Geometry check sheet. Reference: the model listing, model coordinates, mm. A direction names the side the tool comes from. Round coordinates to 2 decimals unless told otherwise and drop trailing zeros. Loops run counter-clockwise (first coordinate to the right, second up) from the corner with the lowest first, then second, coordinate; pieces in that order, holes last. Notation, with made-up numbers: M 27.25,-4.75 L 40.25,-4.75 A17 cw 40.25,28.25 Z; hole C 1.5,-36 d10. An arc over 180 degrees is marked long. Use one line per item in the form item = value. Start each with the question number.
1. Cross-section at B-B (x = 10.5). State how many separate pieces and enclosed holes the cut face has, then the cut area to 3 significant figures.
2. Set-up check for faces 1 (the cylindrical face through (10.563, -12.797, 35.846)), 2 (the cylindrical face through (8, 5, 46)): record each of +Z, -Z, +X, -X, +Y, -Y from which the full face is reachable in a straight line by a thin tool's end or side.
3. Material ranges on line 1 (Z direction, x = 8.5, y = 27.55); line 2 (Z direction, x = 6, y = 4.95); line 3 (Y direction, x = 8, z = 3), recorded low to high.
4. Go/stop test with flat-tipped pins: pin 1 (2.5 mm diameter, centred on y = -107.55, z = -94, fed in from +X); pin 2 (7.5 mm diameter, centred on x = 5, z = 51.5, fed in from -Y); pin 3 (7.5 mm diameter, centred on y = -18, z = 42.5, fed in from +X). Record where each tip stops, or that it passes through.
5. Draft check along Z on faces 3 (the flat face through (7, 0, 104)), 4 (the flat face through (7, -35.05, 24)), 5 (the cylindrical face through (10.94, -105.07, -79.33)). Enter one of: pulls with the +Z half, pulls with the -Z half, needs draft (parallel to the pull), parting line crosses it, or undercut.
6. Cross-section at C-C (y = -69.5). Record the boundary of the cut face in (x, z), then the cut area to 3 significant figures.
7. Cross-section at A-A (z = -67). Record the boundary of the cut face in (x, y), then the cut area to 3 significant figures.
```python
from build123d import *

# Parameters (mm, degrees)
SKETCH1_W                                            = 208
SKETCH1_H                                            = 70.1
BOSS_EXTRUDE1_DEPTH                                  = 15
CBORE_FOR_M8_HEXAGON_SOCKET_HEAD_CAP_SCR_D           = 9
CBORE_FOR_M8_HEXAGON_SOCKET_HEAD_CAP_SCR_CBORE_D     = 15
CBORE_FOR_M8_HEXAGON_SOCKET_HEAD_CAP_SCR_CBORE_DEPTH = 9
F_6_0MM_BLIND_HOLE_1_AT_2_COUNT                      = 2
F_6_0MM_BLIND_HOLE_1_AT_2_PITCH                      = 40
SKETCH6_W                                            = 15
SKETCH6_H                                            = 44
BOSS_EXTRUDE2_DEPTH                                  = 82
M5_TAPPED_HOLE1_D                                    = 4.2
M5_TAPPED_HOLE1_DEPTH                                = 12.4
M5_TAPPED_HOLE1_TIP                                  = 1.2618073
F_5_0MM_BLIND_HOLE_1_D                               = 5
F_5_0MM_BLIND_HOLE_1_DEPTH                           = 8
F_5_0MM_BLIND_HOLE_1_TIP                             = 1.502151548
M6_TAPPED_HOLE1_D                                    = 5
M6_TAPPED_HOLE1_DEPTH                                = 15
M6_TAPPED_HOLE1_TIP                                  = 1.502151548
F_5_0MM_BLIND_HOLE_2_D                               = 5
F_5_0MM_BLIND_HOLE_2_DEPTH                           = 8
F_5_0MM_BLIND_HOLE_2_TIP                             = 1.502151548
M5_TAPPED_HOLE2_D                                    = 4.2
M5_TAPPED_HOLE2_DEPTH                                = 12.4
M5_TAPPED_HOLE2_TIP                                  = 1.2618073
M8_CLEARANCE_HOLE1_D                                 = 9
F_6_0MM_BLIND_HOLE_2_D                               = 6
FILLET1_R                                            = 5
CHAMFER1_SIZE                                        = 3


with BuildPart() as part:
    # Sketch1 → Boss-Extrude1 (new body)
    with BuildSketch(Plane(origin=(0, 0, 0), x_dir=(0, 0, -1), z_dir=(1, 0, 0))):
        Rectangle(SKETCH1_W, SKETCH1_H)
    extrude(amount=BOSS_EXTRUDE1_DEPTH)

    # CBORE for M8 Hexagon socket head cap screws1 (through all)
    with Locations(Plane(origin=(15, 0, 0), x_dir=(0, 0, -1), z_dir=(1, 0, 0))):
        with Locations((-43, -15.05), (-3, -15.05)):
            CounterBoreHole(CBORE_FOR_M8_HEXAGON_SOCKET_HEAD_CAP_SCR_D / 2, CBORE_FOR_M8_HEXAGON_SOCKET_HEAD_CAP_SCR_CBORE_D / 2, CBORE_FOR_M8_HEXAGON_SOCKET_HEAD_CAP_SCR_CBORE_DEPTH)

    # Sketch5 → Ø6.0mm blind hole 1 (revolve, cut)
    with BuildSketch(Plane(origin=(15, 4.95, 43), x_dir=(0, 0, -1), z_dir=(0, 1, 0))):
        Polygon((0, 0), (0, 15), (3.25, 15), (3, 14.75), (3, 0.25), (3.25, 0), align=None)
    f_6_0mm_blind_hole_1 = revolve(axis=Axis((21.35, 4.95, 43), (-1, 0, 0)), mode=Mode.SUBTRACT)

    # Ø6.0mm blind hole 1 at 2: Ø6.0mm blind hole 1 ×2
    with Locations(*[(0, 0, -i * F_6_0MM_BLIND_HOLE_1_AT_2_PITCH) for i in range(1, F_6_0MM_BLIND_HOLE_1_AT_2_COUNT)]):
        add(f_6_0mm_blind_hole_1, mode=Mode.SUBTRACT)

    # Sketch6 → Boss-Extrude2 (add)
    with BuildSketch(Plane.XZ.offset(35.05)):
        with Locations((7.5, -82)):
            Rectangle(SKETCH6_W, SKETCH6_H)
    extrude(amount=BOSS_EXTRUDE2_DEPTH)

    # M5 Tapped Hole1
    with Locations(Plane(origin=(15, 0, 0), x_dir=(0, 0, -1), z_dir=(1, 0, 0))):
        with Locations((94, -107.55), (94, -52.55)):
            Hole(M5_TAPPED_HOLE1_D / 2, depth=M5_TAPPED_HOLE1_DEPTH)
            with Locations((0, 0, -(M5_TAPPED_HOLE1_DEPTH + M5_TAPPED_HOLE1_TIP / 2))):  # 118° drill point
                Cone(0, M5_TAPPED_HOLE1_D / 2, M5_TAPPED_HOLE1_TIP, mode=Mode.SUBTRACT)

    # Ø5.0mm blind hole 1
    with Locations(Plane(origin=(15, 0, 0), x_dir=(0, 0, -1), z_dir=(1, 0, 0))):
        with Locations((79, -52.55), (79, -107.55)):
            Hole(F_5_0MM_BLIND_HOLE_1_D / 2, depth=F_5_0MM_BLIND_HOLE_1_DEPTH)
            with Locations((0, 0, -(F_5_0MM_BLIND_HOLE_1_DEPTH + F_5_0MM_BLIND_HOLE_1_TIP / 2))):  # 118° drill point
                Cone(0, F_5_0MM_BLIND_HOLE_1_D / 2, F_5_0MM_BLIND_HOLE_1_TIP, mode=Mode.SUBTRACT)

    # M6 Tapped Hole1
    with Locations(Plane(origin=(15, 0, 0), x_dir=(0, 0, -1), z_dir=(1, 0, 0))):
        with Locations((-76.5, 27.55), (-36.5, 27.55)):
            Hole(M6_TAPPED_HOLE1_D / 2, depth=M6_TAPPED_HOLE1_DEPTH)
            with Locations((0, 0, -(M6_TAPPED_HOLE1_DEPTH + M6_TAPPED_HOLE1_TIP / 2))):  # 118° drill point
                Cone(0, M6_TAPPED_HOLE1_D / 2, M6_TAPPED_HOLE1_TIP, mode=Mode.SUBTRACT)

    # Ø5.0mm blind hole 2
    with Locations(Plane(origin=(15, 0, 0), x_dir=(0, 0, -1), z_dir=(1, 0, 0))):
        with Locations((-96.5, 27.55), (-16.5, 27.55)):
            Hole(F_5_0MM_BLIND_HOLE_2_D / 2, depth=F_5_0MM_BLIND_HOLE_2_DEPTH)
            with Locations((0, 0, -(F_5_0MM_BLIND_HOLE_2_DEPTH + F_5_0MM_BLIND_HOLE_2_TIP / 2))):  # 118° drill point
                Cone(0, F_5_0MM_BLIND_HOLE_2_D / 2, F_5_0MM_BLIND_HOLE_2_TIP, mode=Mode.SUBTRACT)

    # M5 Tapped Hole2
    with Locations(Plane(origin=(15, 0, 0), x_dir=(0, 0, -1), z_dir=(1, 0, 0))):
        with Locations((-96.5, 2.05), (-16.5, 2.05)):
            Hole(M5_TAPPED_HOLE2_D / 2, depth=M5_TAPPED_HOLE2_DEPTH)
            with Locations((0, 0, -(M5_TAPPED_HOLE2_DEPTH + M5_TAPPED_HOLE2_TIP / 2))):  # 118° drill point
                Cone(0, M5_TAPPED_HOLE2_D / 2, M5_TAPPED_HOLE2_TIP, mode=Mode.SUBTRACT)

    # M8 Clearance Hole1 (through all)
    with Locations(Plane(origin=(15, 0, 0), x_dir=(0, 0, -1), z_dir=(1, 0, 0))):
        with Locations((67, -30.05), (97, -30.05), (67, 19.95), (97, 19.95)):
            Hole(M8_CLEARANCE_HOLE1_D / 2)

    # Ø6.0mm blind hole 2 (through all)
    with Locations(Plane(origin=(15, 0, 0), x_dir=(0, 0, -1), z_dir=(1, 0, 0))):
        with Locations((82, -30.05), (82, 19.95)):
            Hole(F_6_0MM_BLIND_HOLE_2_D / 2)

    # Fillet1
    fillet1_edges = [part.edges().sort_by_distance(p)[0] for p in [
        (7.5, -35.05, -60),
    ]]
    fillet(fillet1_edges, radius=FILLET1_R)

    # Chamfer1
    chamfer1_edges = [part.edges().sort_by_distance(p)[0] for p in [
        (7.5, -117.05, -104),
        (7.5, -117.05, -60),
        (7.5, -35.05, 104),
        (7.5, 35.05, 104),
        (7.5, 35.05, -104),
    ]]
    chamfer(chamfer1_edges, length=CHAMFER1_SIZE)


solid = part.part
```
Reported:
q1.separate_pieces = 1
q1.enclosed_holes = 20
q1.area = 17,300 mm²
q2.face_1 = +X
q2.face_2 = +X, -X
q3.line_1 = -104 to 14, 19 to 34, 39 to 74, 79 to 94, 99 to 104
q3.line_2 = -104 to 0, 6 to 40, 46 to 104
q3.line_3 = -35.05 to -22.55, -7.55 to 1.95, 7.95 to 35.05
q4.pin_1 = 2.09
q4.pin_2 = -35.05
q4.pin_3 = 6
q5.face_3 = pulls with the +Z half
q5.face_4 = needs draft
q5.face_5 = undercut
q6.outline = M 0,-104 L 15,-104 L 15,-60 L 0,-60 Z
q6.area = 660 mm²
q7.outline = M 0,-117.05 L 15,-117.05 L 15,-34.55 L 0,-34.55 Z; M 0,-25.55 L 15,-25.55 L 15,15.45 L 0,15.45 Z; M 0,24.45 L 15,24.45 L 15,35.05 L 0,35.05 Z
q7.area = 2,010 mm²
